```python
from build123d import *

# Parameters (mm, degrees)
EXTRUDE_1_DEPTH          = 12.5
HOLE_WIZARD_M14_1_D      = 12
HOLE_WIZARD_M14_1_DEPTH  = 18
SKETCH_7_W               = 66
SKETCH_7_H               = 25
EXTRUDE_2_DEPTH          = 12
CUT_EXTRUDE_5_DEPTH      = 156.608483059
CUT_EXTRUDE_5_DEPTH_BACK = 156.608483059
SKETCH_12_W              = 30
SKETCH_12_H              = 25


with BuildPart() as part:
    # 草图1 → 凸台-拉伸1 (new, symmetric)
    with BuildSketch(Plane.XY):
        Polygon((-33, -150), (-15, -150), (-15, -112.904160338), (0, -112.904160338), (15, -112.904160338), (15, -150), (33, -150), (33, 90), (15, 90), (-15, 90), (-33, 90), align=None)
    extrude(amount=EXTRUDE_1_DEPTH, both=True)

    # M14 螺纹孔1
    with Locations(Plane(origin=(33, -131.5, 0.451602972), x_dir=(0, 0, 1), z_dir=(1, 0, 0))):
        with Locations((0, 0)):
            hole_wizard_m14_1 = Hole(HOLE_WIZARD_M14_1_D / 2, depth=HOLE_WIZARD_M14_1_DEPTH)

    # 镜向1: M14 螺纹孔1 across plane
    add(hole_wizard_m14_1.mirror(Plane(origin=(0, 0, 0), x_dir=(0, 0, 1), z_dir=(1, 0, 0))), mode=Mode.SUBTRACT)

    # 草图7 → 凸台-拉伸2 (add)
    with BuildSketch(Plane(origin=(0, 90, 0), x_dir=(1, 0, 0), z_dir=(0, 1, 0))):
        Rectangle(SKETCH_7_W, SKETCH_7_H)
    extrude(amount=EXTRUDE_2_DEPTH)

    # 草图12 → 切除-拉伸5 (cut, two sides: drawn at the far end of the back side and taken through both)
    with BuildSketch(Plane(origin=(0, 0, -12.5), x_dir=(-1, 0, 0), z_dir=(0, 0, -1)).offset(-CUT_EXTRUDE_5_DEPTH_BACK)):
        with Locations((0, 75.204537633)):
            Rectangle(SKETCH_12_W, SKETCH_12_H)
    extrude(amount=CUT_EXTRUDE_5_DEPTH + CUT_EXTRUDE_5_DEPTH_BACK, mode=Mode.SUBTRACT)


solid = part.part
```
Verification items for the finished model (mm, model axes). A direction names the side the tool comes from. Coordinates: 2 decimals unless noted, no trailing zeros. Write each loop counter-clockwise with the first axis right and the second up, starting at its lowest first coordinate (ties: lowest second). Pieces come first, ordered by that corner, then holes. Notation, with made-up numbers: M 25.25,82.25 L 78.25,82.25 A27 ccw 78.25,102.25 Z; hole C -9.75,76 d3. An arc over 180 degrees is marked long. Answer as a JSON object with one key per item and string values. Group by question number.
(1) Cross-section at C-C, the plane x = 9. Record the cut outline in (y, z).
(2) Cross-section at B-B, the plane y = -131.5. Record the cut outline in (x, z).
(3) Release check for a two-part mould opening along Y. For faces 4 (the face through (-33, -26, 0)), 5 (the face through (15, 75, 0)), 6 (the face through (0, 102, 0)) record: +Y half, -Y half, draft (parallel to the pull), parting line (faces both ways), or undercut.
(4) Gauge pin test, flat ends, axial feed: pin 1 (5 mm diameter, centred on x = -1, z = 1, fed in from -Y); pin 2 (12.5 mm diameter, centred on y = -134, z = -4, fed in from +X). Record the tip position at first contact, or that the pin passes through.
(5) Tool access check on faces 1 (the face through (0, -112.904, 0)), 2 (the face through (33, -26, 0)), 3 (the face through (-15, 75, 0)). Record the directions out of +Z, -Z, +X, -X, +Y, -Y that give a thin tool (end or side, any length) a straight path to the whole face; none if there is none.
(6) Material ranges on line 1 (Y direction, x = -14, z = -0.25); line 2 (Z direction, x = 21.25, y = -131.5); line 3 (X direction, y = -125.5, z = 8.5), recorded low to high.
(7) Cross-section at A-A, the plane z = -8.5. Record the cut outline in (x, y), and give its area (3 significant figures).
Reply:
{
 "1": {"outline": "M -112.9,-12.5 L 62.7,-12.5 L 62.7,12.5 L -112.9,12.5 Z; M 87.7,-12.5 L 102,-12.5 L 102,12.5 L 87.7,12.5 Z"},
 "2": {"outline": "M -33,-12.5 L -15,-12.5 L -15,-5.55 L -33,-5.55 Z; M -33,6.45 L -15,6.45 L -15,12.5 L -33,12.5 Z; M 15,-12.5 L 33,-12.5 L 33,-5.55 L 15,-5.55 Z; M 15,6.45 L 33,6.45 L 33,12.5 L 15,12.5 Z"},
 "3": {"face 4": "draft", "face 5": "undercut", "face 6": "+Y half"},
 "4": {"pin 1": "y = -112.9", "pin 2": "x = 33"},
 "5": {"face 1": "+Z, -Z, -Y", "face 2": "+Z, -Z, +X, +Y, -Y", "face 3": "+Z, -Z"},
 "6": {"line 1": "-112.9 to 62.7, 87.7 to 102", "line 2": "-12.5 to -5.55, 6.45 to 12.5", "line 3": "-33 to -15, 15 to 33"},
 "7": {"outline": "M -33,-150 L -15,-150 L -15,-112.9 L 15,-112.9 L 15,-150 L 33,-150 L 33,102 L -33,102 Z; hole M -15,62.7 L 15,62.7 L 15,87.7 L -15,87.7 Z", "area": "14,800 mm²"}
}
